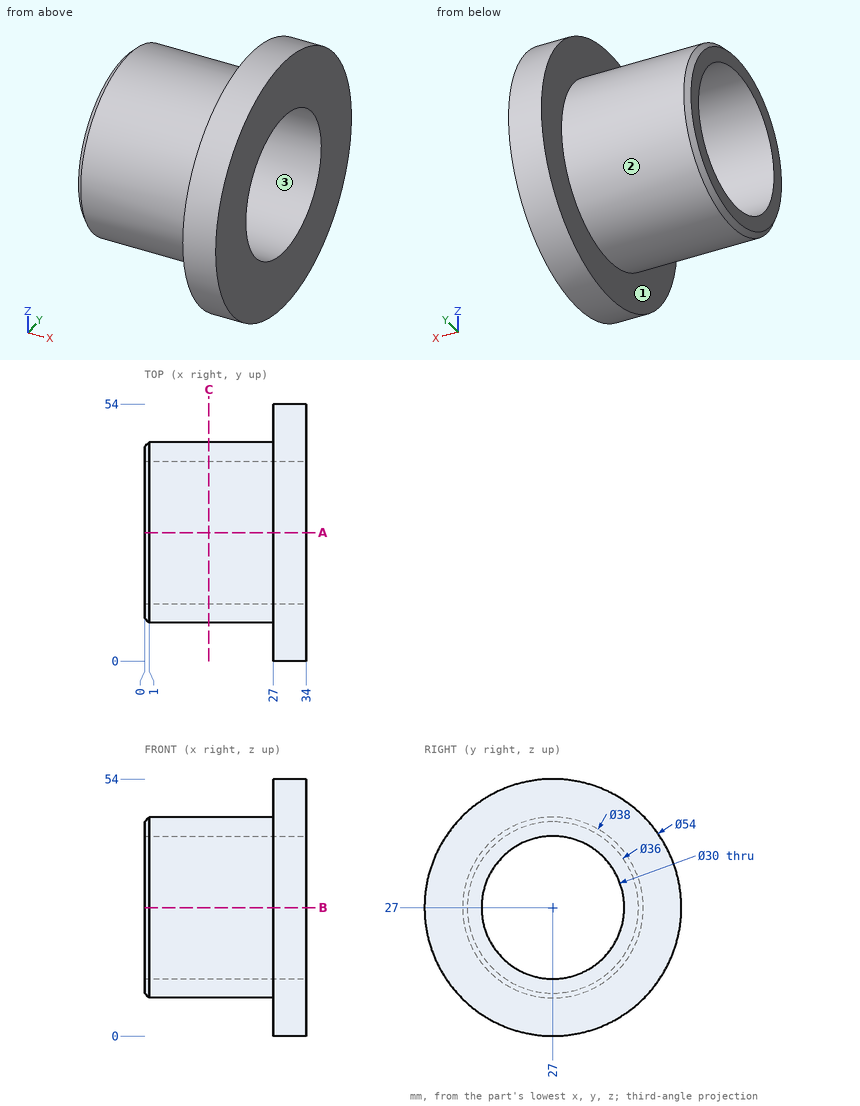
Answer from the drawing. Dimensions are ordinates in mm from the lowest x, y and z of the part. Give positions to 0.01 mm unless a question says otherwise; leave off trailing zeros. Write each loop counter-clockwise with the first axis right and the second up, starting at its lowest first coordinate (ties: lowest second). Pieces come first, ordered by that corner, then holes.
1) Find the intervals of material crossed by L1, parallel to Y at x = 21, z = 27; L2, parallel to X at y = 47, z = 44; L3, parallel to Y at x = 18.5, z = 31.5, in increasing order.
2) Section C-C (x = 13.5) is taken. Write down the section's boundary in (y, z), and give its area (3 significant figures).
3) For a pull along Y with two mould halves and no side action, classify the marked faces 1, 2 and 3 as pulls with the +Y half, pulls with the -Y half, needs draft (parallel to the pull), parting line crosses it, or undercut.
4) Given P1, Ø5, axis at x = 14.5, z = 29.5, coming from the -Y side; P2, Ø6, axis at x = 23, z = 38.5, coming from the -Y side; P3, Ø10, axis at x = 9.5, z = 34.5, coming from the -Y side; P4, Ø1.5, axis at y = 16, z = 17.5, coming from the +X side, each flat-ended and moving along its own axis, determine where each tip first touches the part or whether it passes through.
5) Section A-A (y = 27) is taken. Write down the section's boundary in (x, z), and give its area (3 significant figures).
Response:
1. L1: y = 8 to 12, 42 to 46
1. L2: x = 27 to 34
1. L3: y = 8.54 to 12.69, 41.31 to 45.46
2. outline: circle Ø38 at (27, 27); hole circle Ø30 at (27, 27)
2. area: 427 mm2
3. face 1: needs draft
3. face 2: parting line crosses it
3. face 3: undercut
4. P1: stops at y = 8
4. P2: stops at y = 10.01
4. P3: stops at y = 8.17
4. P4: stops at x = 34
5. outline: (0, 9) - (1, 8) - (27, 8) - (27, 0) - (34, 0) - (34, 12) - (0, 12) - close; (0, 42) - (34, 42) - (34, 54) - (27, 54) - (27, 46) - (1, 46) - (0, 45) - close
5. area: 383 mm2
